```python
from build123d import *

# Parameters (mm, degrees)
FLANGE_PROFILE_SKETCH_R      = 45
FLANGE_PROFILE_SKETCH_R_2    = 5
FLANGE_PROFILE_SKETCH_R_3    = 15
FLANGE_PROFILE_SKETCH_R_4    = 11
MOUNTING_FLANGE_3_LUGS_DEPTH = 14
FLANGE_EDGE_FILLET_R1_R      = 1
BEARING_WALL_SKETCH_R        = 55
BEARING_WALL_SKETCH_R_2      = 45
BEARING_WALL_110_DEPTH       = 23
WALL_START                   = -13
WALL_SLOTS_4X_DEPTH          = 13


with BuildPart() as part:
    # Flange Profile Sketch → Mounting Flange 3 Lugs (new body)
    # profile 1 of 2: a face of its own
    with BuildSketch(Plane(origin=(0, 0, 0), x_dir=(1, 0, 0), z_dir=(0, 1, 0))):
        with BuildLine():
            Line((9.701823617, -72.423761231), (14.543823193, -53.042220984))
            ThreePointArc((14.543823193, -53.042220984), (47.631397208, -27.5), (53.207822442, 13.925790139))
            Line((53.207822442, 13.925790139), (67.571728872, 27.8098549))
            ThreePointArc((67.571728872, 27.8098549), (69.282032303, 40), (57.869905255, 44.613906331))
            Line((57.869905255, 44.613906331), (38.663999249, 39.116430845))
            ThreePointArc((38.663999249, 39.116430845), (0, 55), (-38.663999249, 39.116430845))
            Line((-38.663999249, 39.116430845), (-57.869905255, 44.613906331))
            ThreePointArc((-57.869905255, 44.613906331), (-69.282032303, 40), (-67.571728872, 27.8098549))
            Line((-67.571728872, 27.8098549), (-53.207822442, 13.925790139))
            ThreePointArc((-53.207822442, 13.925790139), (-47.631397208, -27.5), (-14.543823193, -53.042220984))
            Line((-14.543823193, -53.042220984), (-9.701823617, -72.423761231))
            ThreePointArc((-9.701823617, -72.423761231), (0, -80), (9.701823617, -72.423761231))
        make_face()
        Circle(FLANGE_PROFILE_SKETCH_R, mode=Mode.SUBTRACT)
        with Locations(Location((0, -70, 0), (0, 0, 270))):
            Circle(FLANGE_PROFILE_SKETCH_R_2, mode=Mode.SUBTRACT)
        with Locations(Location((-60.621778265, 35, 0), (0, 0, 270))):
            Circle(FLANGE_PROFILE_SKETCH_R_2, mode=Mode.SUBTRACT)
        with Locations(Location((60.621778265, 35, 0), (0, 0, 270))):
            Circle(FLANGE_PROFILE_SKETCH_R_2, mode=Mode.SUBTRACT)
    # profile 2 of 2: a face of its own
    with BuildSketch(Plane(origin=(0, 0, 0), x_dir=(1, 0, 0), z_dir=(0, 1, 0))):
        Circle(FLANGE_PROFILE_SKETCH_R)
        with Locations(Location((0, 0, 0), (0, 0, 270))):
            Circle(FLANGE_PROFILE_SKETCH_R_3, mode=Mode.SUBTRACT)
        with Locations(Location((-25.980762114, -15, 0), (0, 0, 270))):
            Circle(FLANGE_PROFILE_SKETCH_R_4, mode=Mode.SUBTRACT)
        with Locations(Location((25.980762114, -15, 0), (0, 0, 270))):
            Circle(FLANGE_PROFILE_SKETCH_R_4, mode=Mode.SUBTRACT)
        with Locations(Location((0, 30, 0), (0, 0, 270))):
            Circle(FLANGE_PROFILE_SKETCH_R_4, mode=Mode.SUBTRACT)
    extrude(amount=MOUNTING_FLANGE_3_LUGS_DEPTH)

    # Flange Edge Fillet R1
    flange_edge_fillet_r1_edges = [part.edges().sort_by_distance(p)[0] for p in [
        (12.122823405, 14, 62.732991107),
        (60.389775657, 14, -20.867822519),
        (69.282032303, 14, -40),
        (48.266952252, 14, -41.865168588),
        (-48.266952252, 14, -41.865168588),
        (-69.282032303, 14, -40),
        (-60.389775657, 14, -20.867822519),
        (-12.122823405, 14, 62.732991107),
        (0, 14, 80),
    ]]
    fillet(flange_edge_fillet_r1_edges, radius=FLANGE_EDGE_FILLET_R1_R)

    # Bearing Wall Sketch → Bearing Wall Ø110 (add)
    with BuildSketch(Plane(origin=(0, 14, 0), x_dir=(1, 0, 0), z_dir=(0, 1, 0))):
        with Locations(Location((0, 0, 0), (0, 0, 134.666726854))):
            Circle(BEARING_WALL_SKETCH_R)
        with Locations(Location((0, 0, 0), (0, 0, 270))):
            Circle(BEARING_WALL_SKETCH_R_2, mode=Mode.SUBTRACT)
    extrude(amount=BEARING_WALL_110_DEPTH)

    # Wall Slots Sketch → Wall Slots 4x (cut)
    with BuildSketch(Plane(origin=(0, 37, 0), x_dir=(1, 0, 0), z_dir=(0, 1, 0)).offset(WALL_START)):
        with BuildLine():
            ThreePointArc((-44.72135955, -5), (-45, 0), (-44.72135955, 5))
            Line((-44.72135955, 5), (-54.772255751, 5))
            ThreePointArc((-54.772255751, 5), (-55, 0), (-54.772255751, -5))
            Line((-54.772255751, -5), (-44.72135955, -5))
        make_face()
        with BuildLine():
            Line((-5, 54.772255751), (-5, 44.72135955))
            ThreePointArc((-5, 44.72135955), (0, 45), (5, 44.72135955))
            Line((5, 44.72135955), (5, 54.772255751))
            ThreePointArc((5, 54.772255751), (0, 55), (-5, 54.772255751))
        make_face()
        with BuildLine():
            Line((54.772255751, 5), (44.72135955, 5))
            ThreePointArc((44.72135955, 5), (44.930285887, 2.503879016), (45, 0))
            ThreePointArc((45, 0), (44.930285887, -2.503879016), (44.72135955, -5))
            Line((44.72135955, -5), (54.772255751, -5))
            ThreePointArc((54.772255751, -5), (54.943034437, -2.502592028), (55, 0))
            ThreePointArc((55, 0), (54.943034437, 2.502592028), (54.772255751, 5))
        make_face()
        with BuildLine():
            ThreePointArc((5, -44.72135955), (0, -45), (-5, -44.72135955))
            Line((-5, -44.72135955), (-5, -54.772255751))
            ThreePointArc((-5, -54.772255751), (0, -55), (5, -54.772255751))
            Line((5, -54.772255751), (5, -44.72135955))
        make_face()
    extrude(amount=WALL_SLOTS_4X_DEPTH, mode=Mode.SUBTRACT)


solid = part.part
```
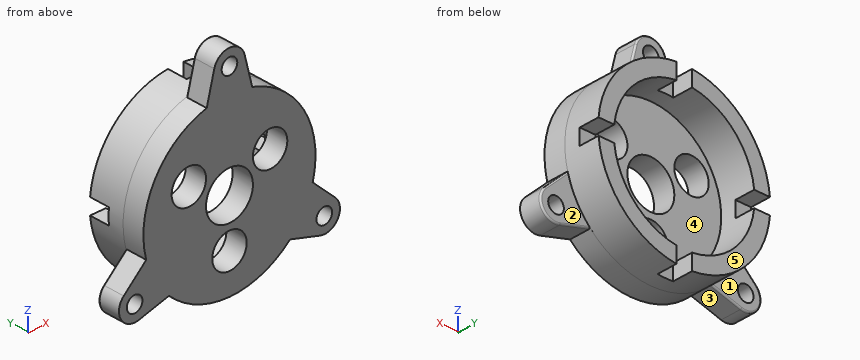
Verification items for the finished model (mm, model axes). Face numbers are marked on the shaded views. A direction names the side the tool comes from. Round coordinates to 2 decimals unless told otherwise and drop trailing zeros. Order: outer loops, then holes, each group sorted by start corner. A loop starts at its lowest first (then second) coordinate and runs counter-clockwise, first axis right, second up. Notation, with made-up numbers: (10.25, -25) -> (66.25, -25) arc R32 cw to (66.25, 8) -> close; hole circle Ø7 at (30, -5). An arc over 180 degrees is marked (long way). Put each result on its own line as item: value. Start each with the question number.
(1) Section check D-D (x = 19.5). Enter the section's corners in (y, z).
(2) Tool access check on the marked faces 1, 2, 3, 4 and 5. Record the directions out of +Z, -Z, +X, -X, +Y, -Y that give a thin tool (end or side, any length) a straight path to the whole face; none if there is none.
(3) Section check A-A (y = 27). Enter the section's corners in (x, z), then the cut area to 3 significant figures.
(4) Depth check by flat-ended pin: pin 1 Ø11 at (x, y) = (-51, 30) entering from +Z; pin 2 Ø1.5 at (y, z) = (18.5, -8) entering from +X; pin 3 Ø8 at (x, y) = (49.5, 30.5) entering from -Z. Enter the tip coordinate at first touch or a pass-through.
(5) Section check C-C (z = 0). Enter the section's corners in (x, y).
(6) Section check B-B (x = 0). Enter the section's corners in (y, z).
(7) Material ranges on line 1 along X through (y, z) = (10, -35); line 2 along X through (y, z) = (32, -29); line 3 along Z through (x, y) = (-57, 11.5), recorded low to high.
Completed:
1. outline: (0, -51.43) -> (37, -51.43) -> (37, -40.56) -> (14, -40.56) -> (14, 6.11) -> (0, 6.11) -> close; (0, 23.89) -> (14, 23.89) -> (14, 40.56) -> (37, 40.56) -> (37, 51.43) -> (0, 51.43) -> close
2. face 1: -Z, -X, +Y
2. face 2: -Z, +X, +Y
2. face 3: -Z, +Y, -Y
2. face 4: +Y
2. face 5: +Z, -Z, +X, -X, +Y
3. outline: (-54.77, -5) arc R55 ccw to (-5, -54.77) -> (-5, -44.72) arc R45 cw to (-44.72, -5) -> close; (-54.77, 5) -> (-44.72, 5) arc R45 cw to (-5, 44.72) -> (-5, 54.77) arc R55 ccw to start; (5, -54.77) arc R55 ccw to (54.77, -5) -> (44.72, -5) arc R45 cw to (5, -44.72) -> close; (5, 44.72) arc R45 cw to (44.72, 5) -> (54.77, 5) arc R55 ccw to (5, 54.77) -> close
3. area: 2,740 mm2
4. pin 1: stops at z = 30.9
4. pin 2: stops at x = 54.52
4. pin 3: stops at z = -30.9
5. outline: (-55, 0) -> (-15, 0) -> (-15, 14) -> (-45, 14) -> (-45, 24) -> (-55, 24) -> close; (15, 0) -> (55, 0) -> (55, 24) -> (45, 24) -> (45, 14) -> (15, 14) -> close
6. outline: (0, -55) -> (24, -55) -> (24, -45) -> (14, -45) -> (14, -41) -> (0, -41) -> close; (0, -19) -> (14, -19) -> (14, -15) -> (0, -15) -> close; (0, 15) -> (14, 15) -> (14, 45) -> (24, 45) -> (24, 55) -> (14, 55) -> (14, 65) -> (0, 65) -> close; (0, 75) -> (14, 75) -> (14, 79) arc R1 ccw to (13, 80) -> (0, 80) -> close
7. line 1: x = -70.62 to -65.62, -55.62 to -9.8, 9.8 to 55.62, 65.62 to 70.62
7. line 2: x = -46.73 to -34.41, 34.41 to 46.73
7. line 3: z = -44.36 to -38.45, -31.55 to -17.59
